from build123d import *

# Parameters (mm, degrees)
SKETCH1_R           = 7.5
BOSS_EXTRUDE1_DEPTH = 4
SKETCH2_R           = 8.5
BOSS_EXTRUDE2_DEPTH = 1
DOME1_FACE_RADIUS   = 8.5
DOME1_HEIGHT        = 3
SKETCH3_R           = 6
CUT_EXTRUDE1_DEPTH  = 4
SCALE1_SCALE        = 0.5


with BuildPart() as part:
    # Sketch1 → Boss-Extrude1 (new body)
    with BuildSketch(Plane(origin=(0, 0, 0), x_dir=(1, 0, 0), z_dir=(0, 1, 0))):
        with Locations(Location((0, 0, 0), (0, 0, 270))):
            Circle(SKETCH1_R)
    extrude(amount=BOSS_EXTRUDE1_DEPTH)

    # Sketch2 → Boss-Extrude2 (add)
    with BuildSketch(Plane(origin=(0, 4, 0), x_dir=(1, 0, 0), z_dir=(0, 1, 0))):
        with Locations(Location((0, 0, 0), (0, 0, 270))):
            Circle(SKETCH2_R)
    extrude(amount=BOSS_EXTRUDE2_DEPTH)

    # Dome1: a dome of height H over a round flat face of radius A is a cap of a sphere of radius (A * A + H * H) / (2 * H)
    dome1_r = (DOME1_FACE_RADIUS * DOME1_FACE_RADIUS + DOME1_HEIGHT * DOME1_HEIGHT) / (2 * DOME1_HEIGHT)
    dome1_base = Plane((0, 5, 0), z_dir=(0, 1, 0))
    with Locations(dome1_base.offset(DOME1_HEIGHT - dome1_r)):
        dome1_ball = Sphere(dome1_r, mode=Mode.PRIVATE)
    add(split(dome1_ball, bisect_by=dome1_base, keep=Keep.TOP, mode=Mode.PRIVATE))

    # Sketch3 → Cut-Extrude1 (cut)
    with BuildSketch(Plane.XZ):
        with Locations(Location((0, 0, 0), (0, 0, 270))):
            Circle(SKETCH3_R)
    extrude(amount=-CUT_EXTRUDE1_DEPTH, mode=Mode.SUBTRACT)


with BuildPart() as part_1:
    # Scale1: scaled about (0, 4.383748239, 0)
    add(part.part.scale(SCALE1_SCALE).moved(Location((0, 2.191874119, 0))))


solid = part_1.part
Verification items for the finished model (mm, model axes). A direction names the side the tool comes from. Give positions to 0.01 mm unless a question says otherwise; leave off trailing zeros. Write each loop counter-clockwise with the first axis right and the second up, starting at its lowest first coordinate (ties: lowest second). Pieces come first, ordered by that corner, then holes. Notation, with made-up numbers: M 31,-29.75 L 73,-29.75 A25 cw 73,-6.75 Z; hole C 19,-7.5 d3. An arc over 180 degrees is marked long. Write item = value, one per line.
(1) Material ranges on line 1 (X direction, y = 3.05, z = 0); line 2 (Z direction, x = -1.25, y = 4); line 3 (Z direction, x = -2, y = 2.75), recorded low to high.
Found:
line_1 = -3.75 to -3, 3 to 3.75
line_2 = -3.54 to -2.73, 2.73 to 3.54
line_3 = -3.17 to -2.24, 2.24 to 3.17
(2) Sectioned sample at A-A (x = 0). Record the cut outline in (y, z).
Found:
outline = M 2.19,-3.75 L 4.19,-3.75 L 4.19,-4.25 L 4.69,-4.25 A6.77 ccw 4.69,4.25 L 4.19,4.25 L 4.19,3.75 L 2.19,3.75 L 2.19,3 L 4.19,3 L 4.19,-3 L 2.19,-3 Z
(3) Go/stop test with flat-tipped pins: pin 1 Ø3 at (x, z) = (0, 1) entering from -Y; pin 2 Ø2 at (y, z) = (5.5, 1) entering from -X. Record where each tip stops, or that it passes through.
Found:
pin_1 = 4.19
pin_2 = -4.23
(4) Sectioned sample at C-C (y = 2.95). Record the cut outline in (x, z).
Found:
outline = C 0,0 d7.5; hole C 0,0 d6
(5) Sectioned sample at D-D (y = 4.4). Record the cut outline in (x, z), then the cut area to 3 significant figures.
Found:
outline = C 0,0 d8.5
area = 56.7 mm2
(6) Draft check along X on faces 1 (the face through (0, 4.192, 0)), 2 (the face through (0.9, 3.18, -2.86)), 3 (the face through (4.214, 4.438, -0.553)), 4 (the face through (-4, 4.192, 0)). Enter one of: released by +X, released by -X, zero draft, split by the parting line, or undercut.
Found:
face_1 = undercut
face_2 = undercut
face_3 = split by the parting line
face_4 = zero draft
(7) Access from +Z, -Z, +X, -X, +Y, -Y to the whole of each face (thin tool, end or side, straight path). Record for faces 5 (the face through (3, 2.192, 1)), 6 (the face through (0.165, 3.178, -3.746)).
Found:
face_5 = +Z, -Z, +X, -X, -Y
face_6 = -Y
(8) Sectioned sample at B-B (z = 0). Record the cut outline in (x, y), then the cut area to 3 significant figures.
Found:
outline = M -4.25,4.19 L -3.75,4.19 L -3.75,2.19 L -3,2.19 L -3,4.19 L 3,4.19 L 3,2.19 L 3.75,2.19 L 3.75,4.19 L 4.25,4.19 L 4.25,4.69 A6.77 ccw -4.25,4.69 Z
area = 16.0 mm2
